The model under review builds one solid part; all positions refer to its coordinate system, in mm. A direction names the side the tool comes from. Round coordinates to 2 decimals unless told otherwise and drop trailing zeros. Write each loop counter-clockwise with the first axis right and the second up, starting at its lowest first coordinate (ties: lowest second). Pieces come first, ordered by that corner, then holes. Notation, with made-up numbers: (71.25, 71) -> (87.25, 71) arc R28 ccw to (87.25, 90) -> close; hole circle Ø2 at (81, 14). An arc over 180 degrees is marked (long way). Return JSON: item names as keys, results as strings. Group by question number.
1. For line 1 along X through (y, z) = (0, -2.75); line 2 along Y through (x, z) = (-11, 0); line 3 along Y through (x, z) = (-11, -4.5), list the stretches that pass through material, from the lowest coordinate up. Write a range as from..to.
2. Clearance check with flat-ended pins moving along their axes: P1, Ø4, axis at x = -88, y = 8, coming from the +Z side; P2, Ø10, axis at x = -27.5, z = -1.5, coming from the -Y side; P3, Ø8, axis at x = -15, z = -5, coming from the +Y side; P4, Ø2.5, axis at x = -11, y = 0, coming from the -Z side. State where each tip first meets the part, or that it passes through.
3. Take a section at C-C, the plane x = -26.5. Write out the cut boundary in (y, z).
4. Tool access review of faces 4 (the flat face through (-113, 0, 0)), 5 (the cylindrical face through (-52.27, -1.73, 7.81)): name each direction out of +Z, -Z, +X, -X, +Y, -Y from which nothing blocks a thin tool from reaching the whole face with its end or side.
5. Take a section at A-A, the plane y = 0. Write out the cut boundary in (x, z).
6. Mouldability with a two-part tool opening along X and no side actions: class faces 1 (the cylindrical face through (-12.6, -1.2, -0.1)), 2 (the flat face through (-105, 2, 8)), 3 (the cylindrical face through (-108.45, -11.99, -0.53)) as pulls with the +X half, pulls with the -X half, needs draft (parallel to the pull), parting line crosses it, or undercut.
7. Take a section at B-B, the plane z = 0. Write out the cut boundary in (x, y), then the cut area to 3 significant figures.
8. Take a section at D-D, the plane x = -11. Write out the cut boundary in (y, z).
from build123d import *

# Parameters (mm, degrees)
CUT_EXTRUDE1_DEPTH      = 115.267230648
CUT_EXTRUDE1_DEPTH_BACK = 115.267230648
SKETCH2_R               = 2
CHAMFER1_SIZE           = 1
CHAMFER2_SIZE           = 1


with BuildPart() as part:
    # Sketch1 → Revolve1 (revolve)
    with BuildSketch(Plane.XY):
        Polygon((0, 0), (-113, 0), (-113, 12), (-105, 12), (-105, 8), (0, 8), align=None)
    revolve(axis=Axis((0, 0, 0), (-1, 0, 0)))

    # Sketch2 → Cut-Extrude1 (cut, two sides: drawn at the far end of the back side and taken through both)
    with BuildSketch(Plane.XY.offset(-CUT_EXTRUDE1_DEPTH_BACK)):
        with Locations((-11, 0)):
            Circle(SKETCH2_R)
    extrude(amount=CUT_EXTRUDE1_DEPTH + CUT_EXTRUDE1_DEPTH_BACK, mode=Mode.SUBTRACT)

    # Chamfer1
    chamfer1_edges = [part.edges().sort_by_distance(p)[0] for p in [
        (0, -8, 0),
    ]]
    chamfer(chamfer1_edges, length=CHAMFER1_SIZE)

    # Chamfer2
    chamfer2_edges = [part.edges().sort_by_distance(p)[0] for p in [
        (-113, -12, 0),
    ]]
    chamfer(chamfer2_edges, length=CHAMFER2_SIZE)


solid = part.part
Output:
{
 "1": {"line 1": "x = -113..-13, -9..0", "line 2": "y = -8..-2, 2..8", "line 3": "y = -6.61..-2, 2..6.61"},
 "2": {"P1": "stops at z = 5.29", "P2": "stops at y = -8", "P3": "stops at y = 7.94", "P4": "passes through"},
 "3": {"outline": "circle Ø16 at (0, 0)"},
 "4": {"face 4": "+Z, -Z, -X, +Y, -Y", "face 5": "+X"},
 "5": {"outline": "(-113, -11) -> (-112, -12) -> (-105, -12) -> (-105, -8) -> (-13, -8) -> (-13, 8) -> (-105, 8) -> (-105, 12) -> (-112, 12) -> (-113, 11) -> close; (-9, -8) -> (-1, -8) -> (0, -7) -> (0, 7) -> (-1, 8) -> (-9, 8) -> close"},
 "6": {"face 1": "undercut", "face 2": "pulls with the +X half", "face 3": "needs draft"},
 "7": {"outline": "(-113, -11) -> (-112, -12) -> (-105, -12) -> (-105, -8) -> (-1, -8) -> (0, -7) -> (0, 7) -> (-1, 8) -> (-105, 8) -> (-105, 12) -> (-112, 12) -> (-113, 11) -> close; hole circle Ø4 at (-11, 0)", "area": "1,860 mm^2"},
 "8": {"outline": "(-2, -7.75) -> (-2, 7.75) arc R8 ccw to start; (2, -7.75) arc R8 ccw to (2, 7.75) -> close"}
}
